Design review of the part built by this model. Coordinates are the model's own, in mm. A direction names the side the tool comes from. Coordinates: 2 decimals unless noted, no trailing zeros. Write each loop counter-clockwise with the first axis right and the second up, starting at its lowest first coordinate (ties: lowest second). Pieces come first, ordered by that corner, then holes. Notation, with made-up numbers: (52, 4.25) -> (70, 4.25) arc R21 cw to (70, 17.25) -> close; hole circle Ø3 at (5.5, 32). An arc over 180 degrees is marked (long way). Write item = value, one per line. Start each with the question number.
```python
from build123d import *

# Parameters (mm, degrees)
SKETCH_2_W                   = 236
SKETCH_2_H                   = 14
EXTRUDE_1_DEPTH              = 48
HOLE_WIZARD_M6_1_D           = 6.6
HOLE_WIZARD_M6_1_DEPTH       = 14
HOLE_WIZARD_M6_1_CBORE_D     = 11
HOLE_WIZARD_M6_1_CBORE_DEPTH = 6.4
HOLE_WIZARD_M6_1_TIP         = 1.982840043
CHAMFER_1_SIZE               = 5
HOLE_WIZARD_M6_2_D           = 6.6
HOLE_WIZARD_M6_2_DEPTH       = 14
HOLE_WIZARD_M6_2_CBORE_D     = 11
HOLE_WIZARD_M6_2_CBORE_DEPTH = 6.4
HOLE_WIZARD_M6_2_TIP         = 1.982840043
HOLE_WIZARD_M6_1_2_D         = 6.6


with BuildPart() as part:
    # 草图2 → 凸台-拉伸1 (new body)
    with BuildSketch(Plane.XY):
        with Locations((118, -7)):
            Rectangle(SKETCH_2_W, SKETCH_2_H)
    extrude(amount=EXTRUDE_1_DEPTH)

    # Hole Wizard M6 _1
    with Locations(Plane(origin=(0, -14, 0), x_dir=(-1, 0, 0), z_dir=(0, -1, 0))):
        with Locations((-224.5, -6.5), (-189.5, -6.5), (-189.5, -41.5), (-224.5, -41.5), (-11.5, -41.5), (-46.5, -41.5), (-46.5, -6.5), (-11.5, -6.5)):
            CounterBoreHole(HOLE_WIZARD_M6_1_D / 2, HOLE_WIZARD_M6_1_CBORE_D / 2, HOLE_WIZARD_M6_1_CBORE_DEPTH, depth=HOLE_WIZARD_M6_1_DEPTH)
            with Locations((0, 0, -(HOLE_WIZARD_M6_1_DEPTH + HOLE_WIZARD_M6_1_TIP / 2))):  # 118° drill point
                Cone(0, HOLE_WIZARD_M6_1_D / 2, HOLE_WIZARD_M6_1_TIP, mode=Mode.SUBTRACT)

    # 倒角1
    chamfer_1_edges = [part.edges().sort_by_distance(p)[0] for p in [
        (236, -7, 48),
        (0, -7, 48),
        (236, -7, 0),
        (0, -7, 0),
    ]]
    chamfer(chamfer_1_edges, length=CHAMFER_1_SIZE)

    # M6 六角凹头螺钉的柱形沉头孔2
    with Locations(Plane(origin=(0, 0, 0), x_dir=(1, 0, 0), z_dir=(0, 1, 0))):
        with Locations((75.5, -10), (160.5, -10), (75.5, -38), (160.5, -38)):
            CounterBoreHole(HOLE_WIZARD_M6_2_D / 2, HOLE_WIZARD_M6_2_CBORE_D / 2, HOLE_WIZARD_M6_2_CBORE_DEPTH, depth=HOLE_WIZARD_M6_2_DEPTH)
            with Locations((0, 0, -(HOLE_WIZARD_M6_2_DEPTH + HOLE_WIZARD_M6_2_TIP / 2))):  # 118° drill point
                Cone(0, HOLE_WIZARD_M6_2_D / 2, HOLE_WIZARD_M6_2_TIP, mode=Mode.SUBTRACT)

    # Hole Wizard M6 _1 2 (through all)
    with Locations(Plane(origin=(0, 0, 0), x_dir=(1, 0, 0), z_dir=(0, 1, 0))):
        with Locations((101, -18.5), (135, -18.5)):
            Hole(HOLE_WIZARD_M6_1_2_D / 2)


solid = part.part
```
(1) For pin 1 Ø5.5 at (x, z) = (189.5, 41.5) entering from +Y; pin 2 Ø7.5 at (x, z) = (224.5, 6.5) entering from -Y, all flat-tipped, find the tip position at first contact; note any pin that passes through.
(2) For faces 4 (the face through (234, -7, 45)), 5 (the face through (160, -6.4, 14)), 6 (the face through (51.995, -10.845, 41.258)), list the 3-axis set-ups (+Z, -Z, +X, -X, +Y, -Y) from which the entire face can be reached by the end or side of a thin tool; tool diameter is ignored.
(3) Take a section at A-A, the plane x = 75.5. State the section outline as (y, z) points.
(4) Mouldability with a two-part tool opening along X and no side actions: class faces 1 (the face through (116, -7, 0)), 2 (the face through (3, -7, 2)), 3 (the face through (78.8, -10.3, 9.9)) as pulls with the +X half, pulls with the -X half, needs draft (parallel to the pull), parting line crosses it, or undercut.
(5) Take a section at B-B, the plane x = 101. State the section outline as (y, z) points, then the cut area to 3 significant figures.
(6) For line 1 (X direction, y = -8.75, z = 41.5); line 2 (Z direction, x = 224.5, y = -3); line 3 (X direction, y = -2, z = 38), list the stretches that pass through material, from the lowest coordinate up.
(7) Take a section at C-C, the plane y = -3.5. Count the separate pieces of the cut face and the enclosed holes in it, then the cut area to 3 significant figures.
Report:
q1.pin_1 = through
q1.pin_2 = -7.6
q2.face_4 = +Z, +X, +Y, -Y
q2.face_5 = +Y
q2.face_6 = -Y
q3.outline = (-14, 0) -> (0, 0) -> (0, 4.5) -> (-6.4, 4.5) -> (-6.4, 6.7) -> (-14, 6.7) -> close; (-14, 13.3) -> (-6.4, 13.3) -> (-6.4, 15.5) -> (0, 15.5) -> (0, 32.5) -> (-6.4, 32.5) -> (-6.4, 34.7) -> (-14, 34.7) -> close; (-14, 41.3) -> (-6.4, 41.3) -> (-6.4, 43.5) -> (0, 43.5) -> (0, 48) -> (-14, 48) -> close
q4.face_1 = needs draft
q4.face_2 = pulls with the -X half
q4.face_3 = undercut
q5.outline = (-14, 0) -> (0, 0) -> (0, 15.2) -> (-14, 15.2) -> close; (-14, 21.8) -> (0, 21.8) -> (0, 48) -> (-14, 48) -> close
q5.area = 580 mm2
q6.line_1 = 0 to 6, 17 to 41, 52 to 184, 195 to 219, 230 to 236
q6.line_2 = 0 to 3.2, 9.8 to 38.2, 44.8 to 48
q6.line_3 = 0 to 70, 81 to 155, 166 to 236
q7.separate_pieces = 1
q7.enclosed_holes = 14
q7.area = 10,600 mm2
